Input: dimensioned drawing with shaded views. Units: mm. Origin: part minimum x, y, z. Give positions to 0.01 mm unless a question says otherwise; leave off trailing zeros. Order: outer loops, then holes, each group sorted by start corner. A loop starts at its lowest first (then second) coordinate and runs counter-clockwise, first axis right, second up.
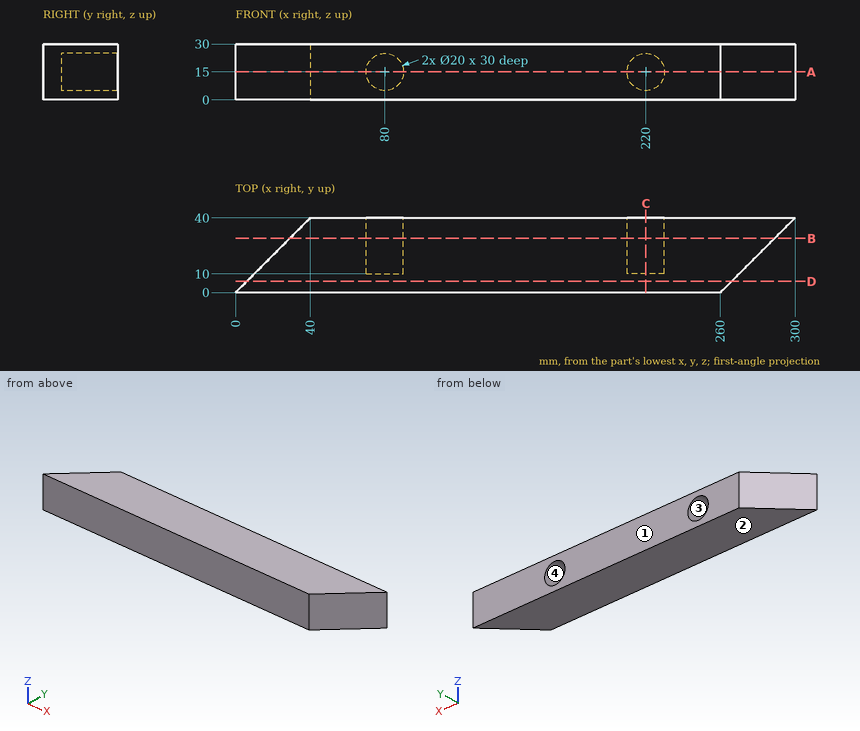
1) Draft query along Z for the marked faces 1, 2, 3 and 4. Return one class per face: +Z half, -Z half, draft (parallel to the pull), parting line (faces both ways), or undercut.
Report:
face 1: draft
face 2: -Z half
face 3: undercut
face 4: undercut
2) Section query A-A, the plane z = 15. Return the cut outline in (x, y).
Report:
outline: (0, 0) - (260, 0) - (300, 40) - (230, 40) - (230, 10) - (210, 10) - (210, 40) - (90, 40) - (90, 10) - (70, 10) - (70, 40) - (40, 40) - close
3) Section query C-C, the plane x = 220. Return the cut outline in (y, z).
Report:
outline: (0, 0) - (40, 0) - (40, 5) - (10, 5) - (10, 25) - (40, 25) - (40, 30) - (0, 30) - close
4) Material intervals for L1, parallel to X at y = 20.5, z = 6; L2, parallel to X at y = 38.5, z = 11.5; L3, parallel to Z at x = 80, y = 33, sorted ascending.
Report:
L1: x = 20.5 to 75.64, 84.36 to 215.64, 224.36 to 280.5
L2: x = 38.5 to 70.63, 89.37 to 210.63, 229.37 to 298.5
L3: z = 0 to 5, 25 to 30
5) Pin query (flat end, axial travel): pin 1 (6 mm diameter, centred on x = 77, z = 12.5, fed in from +Y); pin 2 (3 mm diameter, centred on y = 32, z = 13, fed in from -X); pin 3 (10 mm diameter, centred on y = 28, z = 15, fed in from -X). Return the tip coordinate at first contact, or that it passes through.
Report:
pin 1: stops at y = 10
pin 2: stops at x = 30.5
pin 3: stops at x = 23
6) Section query B-B, the plane y = 29. Return the cut outline in (x, z), and give its area (3 significant figures).
Report:
outline: (29, 0) - (289, 0) - (289, 30) - (29, 30) - close; hole circle Ø20 at (80, 15); hole circle Ø20 at (220, 15)
area: 7,170 mm2
7) Section query D-D, the plane y = 6. Return the cut outline in (x, z), and give its area (3 significant figures).
Report:
outline: (6, 0) - (266, 0) - (266, 30) - (6, 30) - close
area: 7,800 mm2
